```python
from build123d import *

# Parameters (mm, degrees)
SKETCH2_R           = 6
CUT_EXTRUDE1_DEPTH  = 59.523499554
SKETCH3_R           = 14.1
SKETCH3_R_2         = 14
CUT_EXTRUDE2_DEPTH  = 3
CUT_EXTRUDE3_START  = -3
SKETCH4_R           = 14.1
SKETCH4_R_2         = 14
CUT_EXTRUDE3_DEPTH  = 3
SKETCH5_R           = 6
BOSS_EXTRUDE1_DEPTH = 45
SKETCH6_R           = 9
BOSS_EXTRUDE2_DEPTH = 8


with BuildPart() as part:
    # Sketch1 → Revolve1 (revolve)
    with BuildSketch(Plane.XY, mode=Mode.PRIVATE) as revolve1_sk:
        with BuildLine():
            Line((0, 0), (0, 40))
            Line((0, 40), (2, 40))
            Line((2, 40), (5.047051836, 24.51725234))
            ThreePointArc((5.047051836, 24.51725234), (7.5, 22.5), (9.952948164, 24.51725234))
            Line((9.952948164, 24.51725234), (13, 40))
            Line((13, 40), (15, 40))
            Line((15, 40), (15, 0))
            Line((15, 0), (0, 0))
        make_face()
    revolve(revolve1_sk.sketch.rotate(Axis((0, 0, 0), (1, 0, 0)), 90), axis=Axis((0, 0, 0), (1, 0, 0)))

    # Sketch2 → Cut-Extrude1 (cut, through all)
    with BuildSketch(Plane.ZY):
        Circle(SKETCH2_R)
    extrude(amount=-CUT_EXTRUDE1_DEPTH, mode=Mode.SUBTRACT)

    # Sketch3 → Cut-Extrude2 (cut)
    with BuildSketch(Plane.ZY):
        Circle(SKETCH3_R)
        Circle(SKETCH3_R_2, mode=Mode.SUBTRACT)
    extrude(amount=-CUT_EXTRUDE2_DEPTH, mode=Mode.SUBTRACT)

    # Sketch4 → Cut-Extrude3 (cut)
    with BuildSketch(Plane(origin=(15, 0, 0), x_dir=(0, 0, -1), z_dir=(1, 0, 0)).offset(CUT_EXTRUDE3_START)):
        with Locations(Location((0, 0, 0), (0, 0, 180))):
            Circle(SKETCH4_R)
        with Locations(Location((0, 0, 0), (0, 0, 180))):
            Circle(SKETCH4_R_2, mode=Mode.SUBTRACT)
    extrude(amount=CUT_EXTRUDE3_DEPTH, mode=Mode.SUBTRACT)



with BuildPart() as body_2:
    # Sketch5 → Boss-Extrude1 (new body)
    with BuildSketch(Plane(origin=(15, 0, 0), x_dir=(0, 0, -1), z_dir=(1, 0, 0))):
        with Locations(Location((0, 0, 0), (0, 0, 180))):
            Circle(SKETCH5_R)
    extrude(amount=BOSS_EXTRUDE1_DEPTH)


with BuildPart() as part_1:
    add(part.part)

    add(body_2.part)  # Boss-Extrude2 merges body 2
    # Sketch6 → Boss-Extrude2 (add)
    with BuildSketch(Plane(origin=(15, 0, 0), x_dir=(0, 0, -1), z_dir=(1, 0, 0))):
        with Locations(Location((0, 0, 0), (0, 0, 180))):
            Circle(SKETCH6_R)
    extrude(amount=BOSS_EXTRUDE2_DEPTH)


solid = part_1.part
```
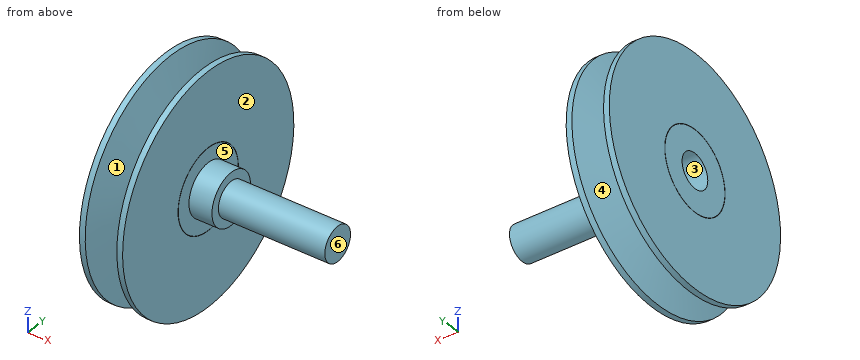
Input: part model. Units: mm. Frame: model coordinates. Face numbers are marked on the shaded views. A direction names the side the tool comes from. Coordinates: 2 decimals unless noted, no trailing zeros. Loops run counter-clockwise (first coordinate to the right, second up) from the corner with the lowest first, then second, coordinate; pieces in that order, holes last. Notation, with made-up numbers: (60.25, 76) - (72.25, 76) arc R18 ccw to (72.25, 107) - close; hole circle Ø8 at (-20, 44). An arc over 180 degrees is marked (long way). Answer in a Markdown table with one row per item.
(1) Mould query, pull axis Y, two halves, no side actions, for the marked faces 1, 2 and 3. Classes: pulls with the +Y half, pulls with the -Y half, needs draft (parallel to the pull), parting line crosses it, or undercut.
Model answer:
| item | result |
|---|---|
| face 1 | parting line crosses it |
| face 2 | needs draft |
| face 3 | undercut |
(2) Set-up query: the marked faces 4, 5 and 6. Return all of +Z, -Z, +X, -X, +Y, -Y with unobstructed straight access to the full face (end or side cutting, diameter ignored); none if empty.
Model answer:
| item | result |
|---|---|
| face 4 | none |
| face 5 | +X |
| face 6 | +Z, -Z, +X, +Y, -Y |
(3) Material intervals for L1, parallel to X at y = -30.5, z = 23.5; L2, parallel to X at y = 11.5, z = 11; L3, parallel to X at y = -11.5, z = -25, sorted ascending. Write a range as from..to.
Model answer:
| item | result |
|---|---|
| L1 | x = 0..2.29, 12.71..15 |
| L2 | x = 0..15 |
| L3 | x = 0..4.46, 10.54..15 |
(4) Cut plane A-A on x = 51. Output: boundary loops of the cut face in (y, z).
Model answer:
| item | result |
|---|---|
| outline | circle Ø12 at (0, 0) |
(5) Pin query (flat end, axial travel): P1, Ø8, axis at y = -22.5, z = -16, coming from the +X side; P2, Ø5, axis at x = 31, y = 6.5, coming from the +Z side; P3, Ø12, axis at x = 49.5, y = -0.5, coming from the +Z side. Return the tip coordinate at first contact, or that it passes through.
Model answer:
| item | result |
|---|---|
| P1 | stops at x = 15 |
| P2 | stops at z = 4.47 |
| P3 | stops at z = 6 |
